The figure shows three views and two pictorial views of one solid part (mm, origin at its lowest corner). Answer the questions. A direction names the side the tool comes from. Round coordinates to 2 decimals unless told otherwise and drop trailing zeros. Loops run counter-clockwise (first coordinate to the right, second up) from the corner with the lowest first, then second, coordinate; pieces in that order, holes last. Notation, with made-up numbers: (73.25, 49.5) -> (85.25, 49.5) arc R37 cw to (85.25, 88.5) -> close; hole circle Ø6 at (-12.5, -35.75). An arc over 180 degrees is marked (long way). Use a Markdown table: item, result. Add a question column.
Q1. Which of the six approach directions +Z, -Z, +X, -X, +Y, -Y give full straight-line access (tool end or side, diameter ignored) to the marked faces 1 and 2?
Q2. Given pin 1 Ø8 at (y, z) = (17.5, 4) entering from +X; pin 2 Ø10 at (x, z) = (27, 18) entering from +Y; pin 3 Ø4 at (x, z) = (67, 8) entering from +Y, each flat-ended and moving along its own axis, determine where each tip first touches the part or whether it passes through.
Q3. Section D-D on x = 14 is taken. Give the vertices of the cut face in (y, z).
Q4. Section C-C on z = 13.25 is taken. Give the vertices of the cut face in (x, y), then the cut area to 3 significant figures.
Q5. For a pull along Y with two mould halves and no side action, classify the marked faces 3, 4 and 5 as released by +Y, released by -Y, zero draft, split by the parting line, or undercut.
Q6. Section A-A on y = 45 is taken. Give the vertices of the cut face in (x, z), then the cut area to 3 significant figures.
Q7. Consider line 1 (Y direction, x = 45, z = 17.75); line 2 (Z direction, x = 22, y = 77.5); line 3 (X direction, y = 31, z = 17.5). Determine where each line is inside the solid, lowest interval first.
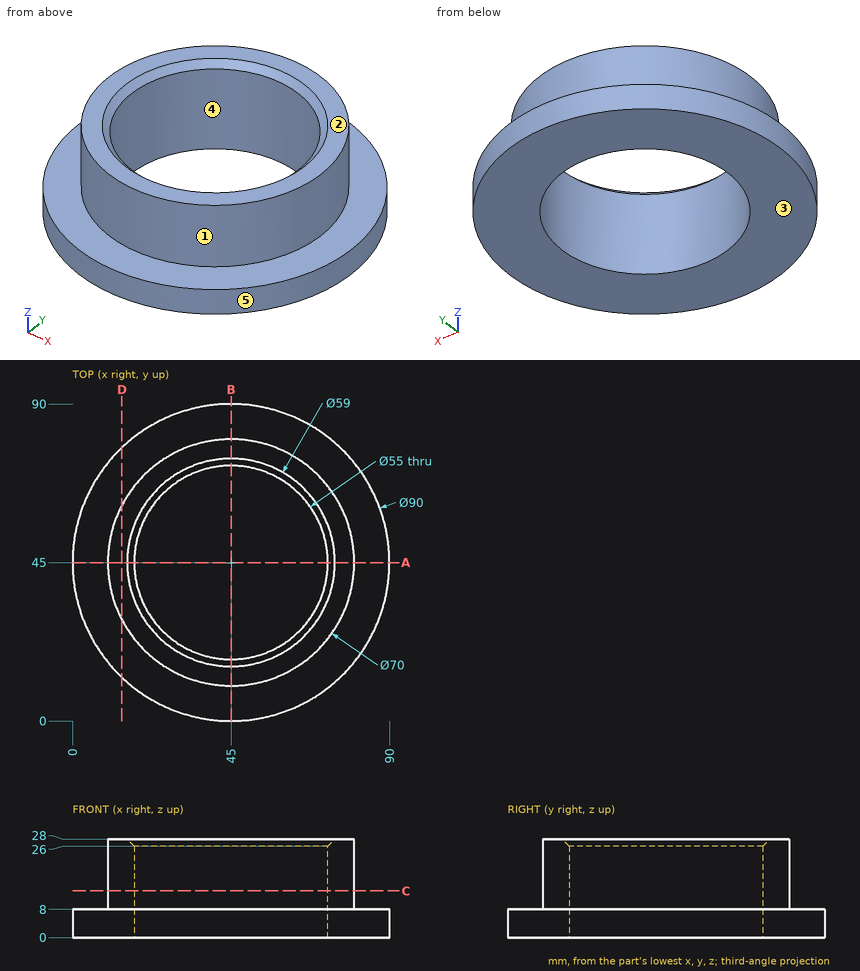
Checked values:
| question | item | result |
|---|---|---|
| 1 | face 1 | +Z |
| 1 | face 2 | +Z, +X, -X, +Y, -Y |
| 2 | pin 1 | stops at x = 83.38 |
| 2 | pin 2 | stops at y = 77.5 |
| 2 | pin 3 | stops at y = 85.31 |
| 3 | outline | (12.38, 0) -> (77.62, 0) -> (77.62, 8) -> (61.25, 8) -> (61.25, 28) -> (28.75, 28) -> (28.75, 8) -> (12.38, 8) -> close |
| 4 | outline | circle Ø70 at (45, 45); hole circle Ø55 at (45, 45) |
| 4 | area | 1,470 mm2 |
| 5 | face 3 | zero draft |
| 5 | face 4 | undercut |
| 5 | face 5 | split by the parting line |
| 6 | outline | (0, 0) -> (17.5, 0) -> (17.5, 26) -> (15.5, 28) -> (10, 28) -> (10, 8) -> (0, 8) -> close; (72.5, 0) -> (90, 0) -> (90, 8) -> (80, 8) -> (80, 28) -> (74.5, 28) -> (72.5, 26) -> close |
| 6 | area | 576 mm2 |
| 7 | line 1 | y = 10 to 17.5, 72.5 to 80 |
| 7 | line 2 | z = 0 to 8 |
| 7 | line 3 | x = 12.92 to 21.33, 68.67 to 77.08 |
